from build123d import *
from OCP.BRepFilletAPI import BRepFilletAPI_MakeChamfer

# Parameters (mm, degrees)
BOSS_EXTRUDE1_DEPTH = 80
CHAMFER1_SIZE       = 1
CHAMFER1_SIZE2      = 0.718015043


with BuildPart() as part:
    # Sketch1 → Boss-Extrude1 (new body)
    with BuildSketch(Plane(origin=(0, 0, 0), x_dir=(0, 0, -1), z_dir=(1, 0, 0))):
        Polygon((0, 0), (0, 47.406641223), (32, 25), (32, 0), align=None)
    extrude(amount=BOSS_EXTRUDE1_DEPTH)

    # Sketch3 → M12 Tapped Hole1 (revolve, cut)
    with BuildSketch(Plane(origin=(12.5, 11, -32), x_dir=(0, 1, 0), z_dir=(1, 0, 0))):
        Polygon((0, 0), (0, 63.064389157), (5.1, 60), (5.1, 0.925), (6.025, 0), align=None)
    m12_tapped_hole1 = revolve(axis=Axis((12.5, 11, -38.35), (0, 0, 1)), mode=Mode.SUBTRACT)

    # Mirror1: M12 Tapped Hole1 across plane
    add(m12_tapped_hole1.mirror(Plane(origin=(40, 0, 0), x_dir=(0, 0, 1), z_dir=(1, 0, 0))), mode=Mode.SUBTRACT)

    # Chamfer1: one chamfer whose edges measure the first distance from different faces: ONE call of the kernel's chamfer builder (chamfer() names one face for all edges)
    chamfer1_edges_1 = [part.edges().sort_by_distance(p)[0] for p in [
        (40, 47.406641223, 0),
    ]]
    chamfer1_side_1 = [part.faces().sort_by_distance(p)[0] for p in [
        (40, 36.203320611, -16),
    ]]
    chamfer1_edges_2 = [part.edges().sort_by_distance(p)[0] for p in [
        (40, 0, -32),
    ]]
    chamfer1 = BRepFilletAPI_MakeChamfer(part.part.solid().wrapped)
    for e in chamfer1_edges_1:
        chamfer1.Add(CHAMFER1_SIZE, CHAMFER1_SIZE2, e.wrapped, chamfer1_side_1[0].wrapped)  # the first distance lies on this face
    for e in chamfer1_edges_2:
        chamfer1.Add(CHAMFER1_SIZE, e.wrapped)
    add(Compound.cast(chamfer1.Shape()), mode=Mode.REPLACE)


solid = part.part
Verification items for the finished model (mm, model axes). Give positions to 0.01 mm unless a question says otherwise; leave off trailing zeros. Write each loop counter-clockwise with the first axis right and the second up, starting at its lowest first coordinate (ties: lowest second). Pieces come first, ordered by that corner, then holes. Notation, with made-up numbers: M 79.5,59 L 88.5,59 A36 ccw 88.5,93 Z; hole C 17,-39 d4. An arc over 180 degrees is marked long. Put each result on its own line as item: value. Start each with the question number.
1. Scan lines: line 1 along X through (y, z) = (11, -22.5); line 2 along Y through (x, z) = (12, -10); line 3 along X through (y, z) = (8.5, -2.5). Record each from-to range of solid material in increasing order. Write a range as [from, to].
2. Go/stop test with flat-tipped pins: pin 1 Ø5 at (x, y) = (29.5, 40) entering from -Z; pin 2 Ø8 at (x, y) = (12.5, 11) entering from -Z. Record where each tip stops, or that it passes through.
3. Section check A-A (x = 12.5). Record the cut outline in (y, z) (3 decimals).
4. Section check B-B (y = 11). Record the cut outline in (x, z) (3 decimals).
5. Section check D-D (x = 34). Record the cut outline in (y, z).
6. Section check C-C (z = -25). Record the cut outline in (x, y), and give its area (3 significant figures).
7. Draft check along Y on faces 1 (the face through (39, 23, 0)), 2 (the face through (10.968, 15.864, -15.755)), 3 (the face through (39, 0, -16)). Enter one of: +Y half, -Y half, draft (parallel to the pull), parting line (faces both ways), or undercut.
Answer list:
1. line 1: [0, 7.4], [17.6, 62.4], [72.6, 80]
1. line 2: [0, 5.92], [16.08, 40.4]
1. line 3: [0, 8.05], [16.95, 63.05], [71.95, 80]
2. pin 1: z = -14.15
2. pin 2: through
3. outline: M 0,-31 L 1,-32 L 4.975,-32 L 5.9,-31.075 L 5.9,0 L 0,0 Z; M 16.1,-31.075 L 17.025,-32 L 25,-32 L 46.833,-0.819 L 46.689,0 L 16.1,0 Z
4. outline: M 0,-32 L 6.475,-32 L 7.4,-31.075 L 7.4,0 L 0,0 Z; M 17.6,-31.075 L 18.525,-32 L 61.475,-32 L 62.4,-31.075 L 62.4,0 L 17.6,0 Z; M 72.6,-31.075 L 73.525,-32 L 80,-32 L 80,0 L 72.6,0 Z
5. outline: M 0,-31 L 1,-32 L 25,-32 L 46.83,-0.82 L 46.69,0 L 0,0 Z
6. outline: M 0,0 L 80,0 L 80,29.9 L 0,29.9 Z; hole C 12.5,11 d10.2; hole C 67.5,11 d10.2
6. area: 2,230 mm2
7. face 1: draft
7. face 2: undercut
7. face 3: -Y half
